```python
from build123d import *

# Parameters (mm, degrees)
JAW_PLATE_12MM_DEPTH   = 6
ROUNDED_END_SKETCH_R   = 6
ROUNDED_END_BOSS_DEPTH = 12
TAPPED_HOLE_M8X1_25_D  = 8


with BuildPart() as part:
    # Jaw Profile Sketch → Jaw Plate 12mm (new, symmetric)
    with BuildSketch(Plane.XY):
        Polygon((0, 0), (-5, 0), (-12, -30), (-12, -74), (0, -74), align=None)
    extrude(amount=JAW_PLATE_12MM_DEPTH, both=True)

    # Rounded End Sketch → Rounded End Boss (add)
    with BuildSketch(Plane(origin=(0, 0, 0), x_dir=(0, 0, -1), z_dir=(1, 0, 0))):
        with Locations((0, -74)):
            Circle(ROUNDED_END_SKETCH_R)
    extrude(amount=-ROUNDED_END_BOSS_DEPTH)

    # Tapped Hole M8x1.25 (through all)
    with Locations(Plane(origin=(0, -74, -0.055848494), x_dir=(0, 0, 1), z_dir=(1, 0, 0))):
        with Locations((0, 0), (0, -35)):
            Hole(TAPPED_HOLE_M8X1_25_D / 2)


solid = part.part
```
Geometry: final body of the model. Coordinates: model frame, mm. Round coordinates to 2 decimals unless told otherwise and drop trailing zeros. Order: outer loops, then holes, each group sorted by start corner. A loop starts at its lowest first (then second) coordinate and runs counter-clockwise, first axis right, second up. Notation, with made-up numbers: (74, 48) -> (104, 48) arc R32 ccw to (104, 87) -> close; hole circle Ø10 at (18, 64). An arc over 180 degrees is marked (long way). Use CSV: the item, a comma, the result in double quotes. Start each with the question number.
1) Section B-B (x = -2.75). Return the cut outline in (y, z).
2) Section D-D (z = -5). Return the cut outline in (x, y), and give its area (3 significant figures).
3) First-contact query: pin 1 Ø5 at (x, z) = (-5, -4.5) entering from -Y; pin 2 Ø5 at (x, z) = (-2, 3.5) entering from -Y. Flat tips, straight axial feed; report the tip coordinate or a pass-through.
4) Material intervals for line 1 along Z through (x, y) = (-4.25, -74); line 2 along Y through (x, z) = (-2.5, 1.25); line 3 along Y through (x, z) = (-4, 1), sorted ascending. Write a range as from..to.
5) Section A-A (y = -39). Return the cut outline in (x, z).
6) Draft query along Z for faces 1 (the face through (-2, 0, 0)), 2 (the face through (-6, -36, 6)), 3 (the face through (-6, -43, 0)). Return one class per face: +Z half, -Z half, draft (parallel to the pull), parting line (faces both ways), or undercut.
7) Section C-C (z = -0.5). Return the cut outline in (x, y).
Returned:
1,outline,"(-74, -6) -> (0, -6) -> (0, 6) -> (-74, 6) arc R6 ccw to start; hole circle Ø8 at (-74, -0.06); hole circle Ø8 at (-39, -0.06)"
2,outline,"(-12, -77.32) -> (0, -77.32) -> (0, 0) -> (-5, 0) -> (-12, -30) -> close"
2,area,"823 mm²"
3,pin 1,"stops at y = -79.66"
3,pin 2,"stops at y = -79.92"
4,line 1,"z = -6..-4.06, 3.94..6"
4,line 2,"y = -79.87..-77.78, -70.22..-42.78, -35.22..0"
4,line 3,"y = -79.92..-77.86, -70.14..-42.86, -35.14..0"
5,outline,"(-12, -6) -> (0, -6) -> (0, -4.06) -> (-12, -4.06) -> close; (-12, 3.94) -> (0, 3.94) -> (0, 6) -> (-12, 6) -> close"
6,face 1,"draft"
6,face 2,"+Z half"
6,face 3,"undercut"
7,outline,"(-12, -79.98) -> (0, -79.98) -> (0, -77.98) -> (-12, -77.98) -> close; (-12, -70.02) -> (0, -70.02) -> (0, -42.98) -> (-12, -42.98) -> close; (-12, -35.02) -> (0, -35.02) -> (0, 0) -> (-5, 0) -> (-12, -30) -> close"
